For this review, take the finished solid that the model builds, in its own axes (mm). Face numbers are marked on the shaded views. A direction names the side the tool comes from. Give positions to 0.01 mm unless a question says otherwise; leave off trailing zeros. Loops run counter-clockwise (first coordinate to the right, second up) from the corner with the lowest first, then second, coordinate; pieces in that order, holes last. Notation, with made-up numbers: (12.25, 30) -> (61.25, 30) arc R15 cw to (61.25, 40) -> close; hole circle Ø11 at (28, 84.5). An arc over 180 degrees is marked (long way). Answer as CSV lines item,"result". Start each with the question number.
Item 1: Add section A-A on y = -13. State the section outline as (x, z) points.
Item 2: Clearance check with flat-ended pins moving along their axes: P1, Ø5, axis at x = 13, y = -13, coming from the -Z side; P2, Ø4, axis at x = 12, y = 13.5, coming from the +Z side; P3, Ø0.8, axis at y = -29, z = -7, coming from the -X side. State where each tip first meets the part, or that it passes through.
Item 3: Add section B-B on y = -5. State the section outline as (x, z) points.
Item 4: The part is to be moulded in two halves that separate along Y. For the marked faces 1, 2 and 3, say which applies: +Y half, -Y half, draft (parallel to the pull), parting line (faces both ways), or undercut.
Item 5: Machinability: for the marked faces 4, 5, 6, 7 and 8, which of the approach directions +Z, -Z, +X, -X, +Y, -Y give a long, thin tool a straight path to every point of the face, cutting with its end or side? Answer none if there is none.
Item 6: For L1, parallel to Z at x = 0, y = 26.5; L2, parallel to Y at x = -12.5, z = 5.5; L3, parallel to Y at x = -13, z = -1.5, list the stretches that pass through material, from the lowest coordinate up. Write a range as from..to.
Item 7: Add section C-C on x = -2.5. State the section outline as (y, z) points, plus the area to 3 significant figures.
```python
from build123d import *

# Parameters (mm, degrees)
SKETCH_1_W                  = 46
SKETCH_1_H                  = 60
EXTRUDE_1_DEPTH             = 8
SKETCH_19_W                 = 142.956519272
SKETCH_19_H                 = 61.410899124
CUT_EXTRUDE_7_DEPTH         = 2
SKETCH_21_W                 = 15
SKETCH_21_H                 = 40
CUT_EXTRUDE_9_DEPTH         = 42.048751504
HOLE_WIZARD_3_0_3_1_D       = 3
HOLE_WIZARD_9_0_9_1_D       = 9
SKETCH_26_W                 = 34.1
SKETCH_26_H                 = 84.411850982
CUT_EXTRUDE_10_DEPTH        = 2
HOLE_WIZARD_3_D             = 4.5
HOLE_WIZARD_3_CBORE_D       = 8
HOLE_WIZARD_3_CBORE_DEPTH   = 7
HOLE_WIZARD_3_2_D           = 4.2
HOLE_WIZARD_3_2_CBORE_D     = 8
HOLE_WIZARD_3_2_CBORE_DEPTH = 7
CHAMFER_2_SIZE              = 3
CHAMFER_1_SIZE              = 3


with BuildPart() as part:
    # 草图1 → 凸台-拉伸1 (new, symmetric)
    with BuildSketch(Plane.XY):
        Rectangle(SKETCH_1_W, SKETCH_1_H)
    extrude(amount=EXTRUDE_1_DEPTH, both=True)

    # 草图19 → 切除-拉伸7 (cut)
    with BuildSketch(Plane.XY.offset(8)):
        with Locations((33.235030531, -50.705449562)):
            Rectangle(SKETCH_19_W, SKETCH_19_H)
    extrude(amount=-CUT_EXTRUDE_7_DEPTH, mode=Mode.SUBTRACT)

    # 草图21 → 切除-拉伸9 (cut, through all)
    with BuildSketch(Plane.XY.offset(8)):
        Rectangle(SKETCH_21_W, SKETCH_21_H)
    extrude(amount=-CUT_EXTRUDE_9_DEPTH, mode=Mode.SUBTRACT)

    # Ø3.0 (3) 直径孔1 (through all)
    with Locations(Plane.XY.offset(8)):
        with Locations((-7.5, 20), (7.5, 20), (-7.5, -20), (7.5, -20)):
            Hole(HOLE_WIZARD_3_0_3_1_D / 2)

    # Ø9.0 (9) 直径孔1 (through all)
    with Locations(Plane(origin=(0, 30, 0), x_dir=(1, 0, 0), z_dir=(0, 1, 0))):
        with Locations((0, -1)):
            Hole(HOLE_WIZARD_9_0_9_1_D / 2)

    # 草图26 → 切除-拉伸10 (cut)
    with BuildSketch(Plane(origin=(0, 0, -8), x_dir=(-1, 0, 0), z_dir=(0, 0, -1))):
        Rectangle(SKETCH_26_W, SKETCH_26_H)
    extrude(amount=-CUT_EXTRUDE_10_DEPTH, mode=Mode.SUBTRACT)

    # Hole Wizard 3 (through all)
    with Locations(Plane(origin=(0, 0, -8), x_dir=(-1, 0, 0), z_dir=(0, 0, -1))):
        with Locations((-15, -25), (15, -25)):
            CounterBoreHole(HOLE_WIZARD_3_D / 2, HOLE_WIZARD_3_CBORE_D / 2, HOLE_WIZARD_3_CBORE_DEPTH)

    # Hole Wizard 3 2 (through all)
    with Locations(Plane.XY.offset(8)):
        with Locations((-13, 13), (13, 13), (-13, -13), (13, -13)):
            CounterBoreHole(HOLE_WIZARD_3_2_D / 2, HOLE_WIZARD_3_2_CBORE_D / 2, HOLE_WIZARD_3_2_CBORE_DEPTH)

    # 倒角2
    chamfer_2_edges = [part.edges().sort_by_distance(p)[0] for p in [
        (-23, 30, 0),
        (23, 30, 0),
    ]]
    chamfer(chamfer_2_edges, length=CHAMFER_2_SIZE)

    # 倒角1
    chamfer_1_edges = [part.edges().sort_by_distance(p)[0] for p in [
        (23, -30, -1),
        (-23, -30, -1),
    ]]
    chamfer(chamfer_1_edges, length=CHAMFER_1_SIZE)


solid = part.part
```
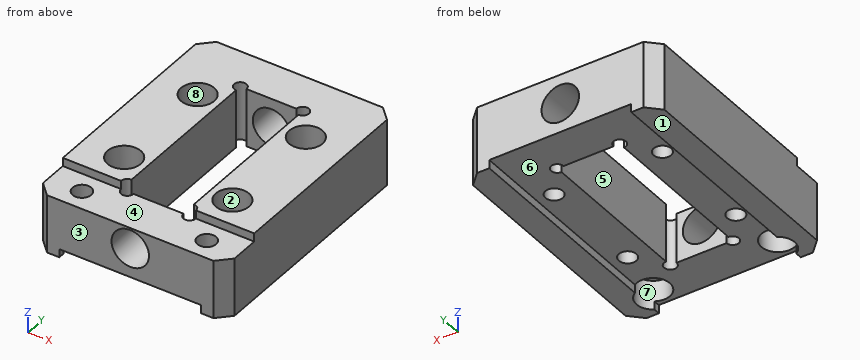
Computed values:
1,outline,"(-23, -8) -> (-17.05, -8) -> (-17.05, -6) -> (-15.1, -6) -> (-15.1, 1) -> (-17, 1) -> (-17, 8) -> (-23, 8) -> close; (-10.9, -6) -> (-7.5, -6) -> (-7.5, 8) -> (-9, 8) -> (-9, 1) -> (-10.9, 1) -> close; (7.5, -6) -> (10.9, -6) -> (10.9, 1) -> (9, 1) -> (9, 8) -> (7.5, 8) -> close; (15.1, -6) -> (17.05, -6) -> (17.05, -8) -> (23, -8) -> (23, 8) -> (17, 8) -> (17, 1) -> (15.1, 1) -> close"
2,P1,"z = -6"
2,P2,"z = 1"
2,P3,"x = -21.4"
3,outline,"(-23, -8) -> (-17.05, -8) -> (-17.05, -6) -> (-7.5, -6) -> (-7.5, 8) -> (-23, 8) -> close; (7.5, -6) -> (17.05, -6) -> (17.05, -8) -> (23, -8) -> (23, 8) -> (7.5, 8) -> close"
4,face 1,"draft"
4,face 2,"undercut"
4,face 3,"-Y half"
5,face 4,"+Z, +X, -X, -Y"
5,face 5,"+Z, -Z"
5,face 6,"-Z, +Y, -Y"
5,face 7,"-Z"
5,face 8,"+Z"
6,L1,"-6..-3.5, 5.5..8"
6,L2,"-30..-16.97, -9.03..9.03, 16.97..30"
6,L3,"-30..-28.46, -21.54..-15.1, -10.9..10.9, 15.1..30"
7,outline,"(-30, -6) -> (-20, -6) -> (-20, -2.74) -> (-30, -2.74) -> close; (-30, 4.74) -> (-20, 4.74) -> (-20, 6) -> (-30, 6) -> close; (20, -6) -> (30, -6) -> (30, -2.74) -> (20, -2.74) -> close; (20, 4.74) -> (30, 4.74) -> (30, 8) -> (20, 8) -> close"
7,area,"110 mm²"
